```python
from build123d import *

# Parameters (mm, degrees)
SPINNER_BODY_DEPTH             = 8
HUB_BOSS_10_SKETCH_R           = 10
HUB_BOSS_10_DEPTH              = 1.5
HUB_BOSS_11_SKETCH_R           = 11
HUB_BOSS_11_DEPTH              = 1.5
HUB_CAP_13_ON_11_BOSS_SKETCH_R = 13
HUB_CAP_13_ON_11_BOSS_DEPTH    = 2
HUB_START                      = 2
HUB_CAP_13_ON_10_BOSS_SKETCH_R = 13
HUB_CAP_13_ON_10_BOSS_DEPTH    = 2
LOBE_HOLES_3X_10_SKETCH_R      = 10
LOBE_HOLES_3X_10_DEPTH         = 8
LOBE_RINGS_3X_10_9_SKETCH_R    = 10
LOBE_RINGS_3X_10_9_SKETCH_R_2  = 9
LOBE_RINGS_3X_10_9_DEPTH       = 8
LOBE_RINGS_3X_9_6_SKETCH_R     = 9
LOBE_RINGS_3X_9_6_SKETCH_R_2   = 6
LOBE_RINGS_3X_9_6_DEPTH        = 8
LOBE_RINGS_3X_6_5_SKETCH_R     = 6
LOBE_RINGS_3X_6_5_SKETCH_R_2   = 5
LOBE_RINGS_3X_6_5_DEPTH        = 8


with BuildPart() as part:
    # Spinner Body Sketch → Spinner Body (new body)
    with BuildSketch(Plane.XY):
        with BuildLine():
            ThreePointArc((-11.816475763, -19.580507354), (-0.317877053, -37.996113041), (12.067302022, -20.164690091))
            ThreePointArc((12.067302022, -20.164690091), (13.213407519, -5.958437932), (25.234931886, 1.697547316))
            ThreePointArc((25.234931886, 1.697547316), (34.838281601, 21.597841349), (12.74333417, 21.35427128))
            ThreePointArc((12.74333417, 21.35427128), (1.248689911, 14.609217628), (-10.684542323, 20.543909185))
            ThreePointArc((-10.684542323, 20.543909185), (-32.475062427, 19.731453355), (-22.869218634, 0.155585152))
            ThreePointArc((-22.869218634, 0.155585152), (-12.326967101, -6.903433276), (-11.816475763, -19.580507354))
        make_face()
    extrude(amount=SPINNER_BODY_DEPTH)

    # Hub Boss Ø10 Sketch → Hub Boss Ø10 (add)
    with BuildSketch(Plane.XY.offset(8)):
        Circle(HUB_BOSS_10_SKETCH_R)
    extrude(amount=HUB_BOSS_10_DEPTH)

    # Hub Boss Ø11 Sketch → Hub Boss Ø11 (add)
    with BuildSketch(Plane(origin=(0, 0, 0), x_dir=(-1, 0, 0), z_dir=(0, 0, -1))):
        with Locations(Location((0, 0, 0), (0, 0, 180))):
            Circle(HUB_BOSS_11_SKETCH_R)
    extrude(amount=HUB_BOSS_11_DEPTH)

    # Hub Cap Ø13 on Ø11 Boss Sketch → Hub Cap Ø13 on Ø11 Boss (add)
    with BuildSketch(Plane(origin=(0, 0, -1.5), x_dir=(-1, 0, 0), z_dir=(0, 0, -1))):
        Circle(HUB_CAP_13_ON_11_BOSS_SKETCH_R)
    extrude(amount=HUB_CAP_13_ON_11_BOSS_DEPTH)

    # Hub Cap Ø13 on Ø10 Boss Sketch → Hub Cap Ø13 on Ø10 Boss (add)
    with BuildSketch(Plane.XY.offset(9.5).offset(HUB_START)):
        with Locations(Location((0, 0, 0), (0, 0, 180))):
            Circle(HUB_CAP_13_ON_10_BOSS_SKETCH_R)
    extrude(amount=-HUB_CAP_13_ON_10_BOSS_DEPTH)

    # Lobe Holes 3xØ10 Sketch → Lobe Holes 3xØ10 (cut)
    with BuildSketch(Plane(origin=(0, 0, 0), x_dir=(-1, 0, 0), z_dir=(0, 0, -1))):
        with Locations((-23.866329129, 14.6253053)):
            Circle(LOBE_HOLES_3X_10_SKETCH_R)
        with Locations((21.316004109, 13.062464118)):
            Circle(LOBE_HOLES_3X_10_SKETCH_R)
        with Locations((0, -25)):
            Circle(LOBE_HOLES_3X_10_SKETCH_R)
    extrude(amount=-LOBE_HOLES_3X_10_DEPTH, mode=Mode.SUBTRACT)

    # Lobe Rings 3xØ10-Ø9 Sketch → Lobe Rings 3xØ10-Ø9 (add)
    # profile 1 of 3: a face of its own
    with BuildSketch(Plane(origin=(0, 0, 0), x_dir=(-1, 0, 0), z_dir=(0, 0, -1))):
        with Locations((-23.866329129, 14.6253053)):
            Circle(LOBE_RINGS_3X_10_9_SKETCH_R)
        with Locations((-23.866329129, 14.6253053)):
            Circle(LOBE_RINGS_3X_10_9_SKETCH_R_2, mode=Mode.SUBTRACT)
    # profile 2 of 3: a face of its own
    with BuildSketch(Plane(origin=(0, 0, 0), x_dir=(-1, 0, 0), z_dir=(0, 0, -1))):
        with Locations((21.316004109, 13.062464118)):
            Circle(LOBE_RINGS_3X_10_9_SKETCH_R)
        with Locations((21.316004109, 13.062464118)):
            Circle(LOBE_RINGS_3X_10_9_SKETCH_R_2, mode=Mode.SUBTRACT)
    # profile 3 of 3: a face of its own
    with BuildSketch(Plane(origin=(0, 0, 0), x_dir=(-1, 0, 0), z_dir=(0, 0, -1))):
        with Locations((0, -25)):
            Circle(LOBE_RINGS_3X_10_9_SKETCH_R)
        with Locations((0, -25)):
            Circle(LOBE_RINGS_3X_10_9_SKETCH_R_2, mode=Mode.SUBTRACT)
    extrude(amount=-LOBE_RINGS_3X_10_9_DEPTH)

    # Lobe Rings 3xØ9-Ø6 Sketch → Lobe Rings 3xØ9-Ø6 (add)
    # profile 1 of 3: a face of its own
    with BuildSketch(Plane(origin=(0, 0, 0), x_dir=(-1, 0, 0), z_dir=(0, 0, -1))):
        with Locations((-23.866329129, 14.6253053)):
            Circle(LOBE_RINGS_3X_9_6_SKETCH_R)
        with Locations((-23.866329129, 14.6253053)):
            Circle(LOBE_RINGS_3X_9_6_SKETCH_R_2, mode=Mode.SUBTRACT)
    # profile 2 of 3: a face of its own
    with BuildSketch(Plane(origin=(0, 0, 0), x_dir=(-1, 0, 0), z_dir=(0, 0, -1))):
        with Locations((21.316004109, 13.062464118)):
            Circle(LOBE_RINGS_3X_9_6_SKETCH_R)
        with Locations((21.316004109, 13.062464118)):
            Circle(LOBE_RINGS_3X_9_6_SKETCH_R_2, mode=Mode.SUBTRACT)
    # profile 3 of 3: a face of its own
    with BuildSketch(Plane(origin=(0, 0, 0), x_dir=(-1, 0, 0), z_dir=(0, 0, -1))):
        with Locations((0, -25)):
            Circle(LOBE_RINGS_3X_9_6_SKETCH_R)
        with Locations((0, -25)):
            Circle(LOBE_RINGS_3X_9_6_SKETCH_R_2, mode=Mode.SUBTRACT)
    extrude(amount=-LOBE_RINGS_3X_9_6_DEPTH)

    # Lobe Rings 3xØ6-Ø5 Sketch → Lobe Rings 3xØ6-Ø5 (add)
    # profile 1 of 3: a face of its own
    with BuildSketch(Plane(origin=(0, 0, 0), x_dir=(-1, 0, 0), z_dir=(0, 0, -1))):
        with Locations((-23.866329129, 14.6253053)):
            Circle(LOBE_RINGS_3X_6_5_SKETCH_R)
        with Locations((-23.866329129, 14.6253053)):
            Circle(LOBE_RINGS_3X_6_5_SKETCH_R_2, mode=Mode.SUBTRACT)
    # profile 2 of 3: a face of its own
    with BuildSketch(Plane(origin=(0, 0, 0), x_dir=(-1, 0, 0), z_dir=(0, 0, -1))):
        with Locations((21.316004109, 13.062464118)):
            Circle(LOBE_RINGS_3X_6_5_SKETCH_R)
        with Locations((21.316004109, 13.062464118)):
            Circle(LOBE_RINGS_3X_6_5_SKETCH_R_2, mode=Mode.SUBTRACT)
    # profile 3 of 3: a face of its own
    with BuildSketch(Plane(origin=(0, 0, 0), x_dir=(-1, 0, 0), z_dir=(0, 0, -1))):
        with Locations((0, -25)):
            Circle(LOBE_RINGS_3X_6_5_SKETCH_R)
        with Locations((0, -25)):
            Circle(LOBE_RINGS_3X_6_5_SKETCH_R_2, mode=Mode.SUBTRACT)
    extrude(amount=-LOBE_RINGS_3X_6_5_DEPTH)


solid = part.part
```
Input: part model. Units: mm. Frame: model coordinates. A direction names the side the tool comes from. Coordinates: 2 decimals unless noted, no trailing zeros. Write each loop counter-clockwise with the first axis right and the second up, starting at its lowest first coordinate (ties: lowest second). Pieces come first, ordered by that corner, then holes.
1) Section C-C on z = 1.75. Output: boundary loops of the cut face in (x, y).
2) Set-up query: faces 1 (the flat face through (0, 0, 11.5)), 2 (the flat face through (11, 3, -1.5)), 3 (the cylindrical face through (10.316, -7.91, -2.486)), 4 (the cylindrical face through (10.316, 7.91, 10.514)). Return all of +Z, -Z, +X, -X, +Y, -Y with unobstructed straight access to the full face (end or side cutting, diameter ignored); none if empty.
3) Pin query (flat end, axial travel): pin 1 Ø8 at (x, y) = (-23.5, 12.5) entering from -Z; pin 2 Ø4 at (x, z) = (22, 9) entering from -Y; pin 3 Ø11.5 at (x, y) = (-21.32, 13.06) entering from +Z. Return the tip coordinate at first contact, or that it passes through.
4) Material intervals for line 1 along Z through (x, y) = (-11, -1); line 2 along X through (y, z) = (14.5, 3.75); line 3 along Y through (x, z) = (0, 5.5), sorted ascending.
5) Mould query, pull axis X, two halves, no side actions, for faces 5 (the cylindrical face through (-2.17, -9.76, 8.74)), 6 (the cylindrical face through (1.08, -29.88, 3.94)), 7 (the flat face through (10, 3, 8)). Classes: pulls with the +X half, pulls with the -X half, needs draft (parallel to the pull), parting line crosses it, or undercut.
6) Section A-A on x = 0. Output: boundary loops of the cut face in (y, z), and give its area (3 significant figures).
7) Section B-B on y = -28. Output: boundary loops of the cut face in (x, z).
8) Section D-D on y = 3. Output: boundary loops of the cut face in (x, z), and give its area (3 significant figures).
Check result:
1. outline: (-22.87, 0.16) arc R14 cw to (-11.82, -19.58) arc R13 ccw (long way) to (12.07, -20.16) arc R16 cw to (25.23, 1.7) arc R13 ccw (long way) to (12.74, 21.35) arc R14 cw to (-10.68, 20.54) arc R13 ccw (long way) to start; hole circle Ø10 at (-21.32, 13.06); hole circle Ø10 at (0, -25); hole circle Ø10 at (23.87, 14.63)
2. face 1: +Z, +X, -X, +Y, -Y
2. face 2: none
2. face 3: -Z
2. face 4: +Z
3. pin 1: stops at z = 0
3. pin 2: stops at y = 0.34
3. pin 3: stops at z = 8
4. line 1: z = -3.5 to -1.5, 0 to 8, 9.5 to 11.5
4. line 2: x = -34.24 to -26.1, -16.53 to 18.87, 28.86 to 36.87
4. line 3: y = -38 to -30, -20 to 14.62
5. face 5: parting line crosses it
5. face 6: undercut
5. face 7: needs draft
6. outline: (-38, 0) - (-30, 0) - (-30, 8) - (-38, 8) - close; (-20, 0) - (-11, 0) - (-11, -1.5) - (-13, -1.5) - (-13, -3.5) - (13, -3.5) - (13, -1.5) - (11, -1.5) - (11, 0) - (14.62, 0) - (14.62, 8) - (10, 8) - (10, 9.5) - (13, 9.5) - (13, 11.5) - (-13, 11.5) - (-13, 9.5) - (-10, 9.5) - (-10, 8) - (-20, 8) - close
6. area: 508 mm2
7. outline: (-12.65, 0) - (-4, 0) - (-4, 8) - (-12.65, 8) - close; (4, 0) - (12.65, 0) - (12.65, 8) - (4, 8) - close
8. outline: (-29.55, 0) - (-10.58, 0) - (-10.58, -1.5) - (-12.65, -1.5) - (-12.65, -3.5) - (12.65, -3.5) - (12.65, -1.5) - (10.58, -1.5) - (10.58, 0) - (29.68, 0) - (29.68, 8) - (9.54, 8) - (9.54, 9.5) - (12.65, 9.5) - (12.65, 11.5) - (-12.65, 11.5) - (-12.65, 9.5) - (-9.54, 9.5) - (-9.54, 8) - (-29.55, 8) - close
8. area: 635 mm2
